For this review, take the finished solid that the model builds, in its own axes (mm). Face numbers are marked on the shaded views. A direction names the side the tool comes from. Round coordinates to 2 decimals unless told otherwise and drop trailing zeros. Write each loop counter-clockwise with the first axis right and the second up, starting at its lowest first coordinate (ties: lowest second). Pieces come first, ordered by that corner, then holes. Notation, with made-up numbers: (41.25, -30) -> (86.25, -30) arc R30 ccw to (86.25, 5) -> close; hole circle Ø5 at (45, -6). An arc over 180 degrees is marked (long way). Answer as CSV lines item,"result". Start each with the question number.
Item 1: Wall thickness on probe 1 along Y at (x, z) = (101.5, 18); probe 2 along Z at (x, y) = (75, -100); probe 3 along Y at (x, z) = (37, -8): over which ranges is each line inside the solid? List them lowest first. Write a range as from..to.
Item 2: For pin 1 Ø4 at (y, z) = (-101, -11.5) entering from -X; pin 2 Ø12 at (y, z) = (-50.5, -2) entering from -X; pin 3 Ø15 at (y, z) = (-28, 5.5) entering from +X; pin 4 Ø15 at (y, z) = (0, 0) entering from +X, all flat-tipped, find the tip position at first contact; note any pin that passes through.
Item 3: Take a section at B-B on x = 15. Give the boundary of the cut face in (y, z), then the cut area to 3 significant figures.
Item 4: Take a section at D-D on x = 79.5. Give the boundary of the cut face in (y, z), then the cut area to 3 significant figures.
Item 5: Machinability: for the marked faces 5, 6 and 7, which of the approach directions +Z, -Z, +X, -X, +Y, -Y give a long, thin tool a straight path to every point of the face, cutting with its end or side? Answer none if there is none.
Item 6: Take a section at C-C on y = -49. Give the boundary of the cut face in (x, z), then the cut area to 3 significant figures.
Item 7: Take a section at A-A on z = 0. Give the boundary of the cut face in (x, y), then the cut area to 3 significant figures.
Item 8: Mouldability with a two-part tool opening along Y and no side actions: class the marked faces 1, 2, 3 and 4 as +Y half, -Y half, draft (parallel to the pull), parting line (faces both ways), or undercut.
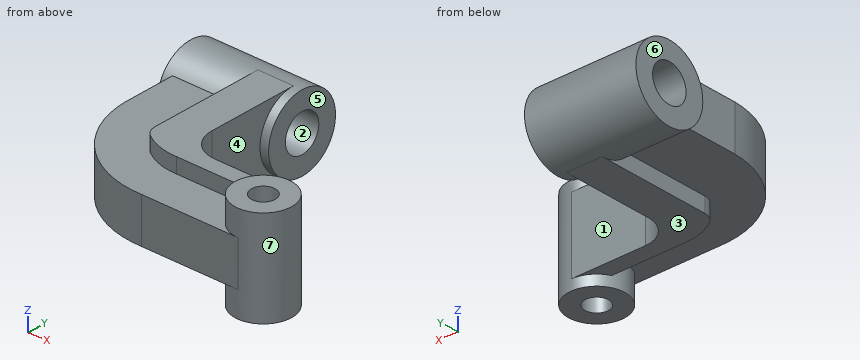
```python
from build123d import *

# Parameters (mm, degrees)
HUB_1_PROFILE_R       = 25
HUB_1_BOSS_75MM_DEPTH = 37.5
HUB_2_PROFILE_R       = 19
HUB_2_BOSS_64MM_DEPTH = 32
CURVED_ARM_WEB_DEPTH  = 15
ARM_FLANGE_DEPTH      = 25
HUB_1_BORE_PROFILE_R  = 12.5
HUB_1_BORE_DEPTH      = 88
HUB_2_BORE_PROFILE_R  = 8
HUB_2_BORE_DEPTH      = 88


with BuildPart() as part:
    # Hub 1 Profile → Hub 1 Boss 75mm (new, symmetric)
    with BuildSketch(Plane(origin=(0, 0, 0), x_dir=(0, 0, -1), z_dir=(1, 0, 0))):
        Circle(HUB_1_PROFILE_R)
    extrude(amount=HUB_1_BOSS_75MM_DEPTH, both=True)



with BuildPart() as body_2:
    # Hub 2 Profile → Hub 2 Boss 64mm (new, symmetric)
    with BuildSketch(Plane.XY):
        with Locations((101.5, -100)):
            Circle(HUB_2_PROFILE_R)
    extrude(amount=HUB_2_BOSS_64MM_DEPTH, both=True)


with BuildPart() as part_1:
    add(part.part)

    add(body_2.part)  # Curved Arm Web merges body 2
    # Curved Arm Profile → Curved Arm Web (add, symmetric)
    with BuildSketch(Plane.XY):
        with BuildLine():
            Line((36.70784585, -119), (101.5, -119))
            ThreePointArc((101.5, -119), (85.489542295, -110.23060331), (84.258248254, -92.017394113))
            Line((84.258248254, -92.017394113), (35.73883627, -92.017394113))
            ThreePointArc((35.73883627, -92.017394113), (23.331450339, -90.456826651), (12.055799796, -85.049581394))
            ThreePointArc((12.055799796, -85.049581394), (8.905598759, -81.472069365), (7.769480814, -76.842642304))
            Line((7.769480814, -76.842642304), (7.769480814, -18.704046106))
            Line((7.769480814, -18.704046106), (-31.61832529, -18.704046106))
            Line((-31.61832529, -18.704046106), (-31.61832529, -25))
            Line((-31.61832529, -25), (-31.61832529, -55.411209028))
            ThreePointArc((-31.61832529, -55.411209028), (-10.624909538, -101.356417889), (36.70784585, -119))
        make_face()
    extrude(amount=CURVED_ARM_WEB_DEPTH, both=True)

    # Arm Flange Profile → Arm Flange (add, symmetric)
    with BuildSketch(Plane.XY):
        with BuildLine():
            Line((31.704445688, -20), (31.704445688, -61))
            ThreePointArc((31.704445688, -61), (37.562310065, -75.142135624), (51.704445688, -81))
            Line((51.704445688, -81), (101.5, -81))
            ThreePointArc((101.5, -81), (91.26939669, -83.989542295), (84.258248254, -92.017394113))
            Line((84.258248254, -92.017394113), (35.73883627, -92.017394113))
            ThreePointArc((35.73883627, -92.017394113), (23.331450339, -90.456826651), (12.055799796, -85.049581394))
            ThreePointArc((12.055799796, -85.049581394), (8.905598759, -81.472069365), (7.769480814, -76.842642304))
            Line((7.769480814, -76.842642304), (7.769480814, -20))
            Line((7.769480814, -20), (7.769480814, 0))
            Line((7.769480814, 0), (31.704445688, 0))
            Line((31.704445688, 0), (31.704445688, -20))
        make_face()
    extrude(amount=ARM_FLANGE_DEPTH, both=True)

    # Hub 1 Bore Profile → Hub 1 Bore (cut)
    with BuildSketch(Plane(origin=(37.5, 0, 0), x_dir=(0, 0, -1), z_dir=(1, 0, 0))):
        Circle(HUB_1_BORE_PROFILE_R)
    extrude(amount=-HUB_1_BORE_DEPTH, mode=Mode.SUBTRACT)

    # Hub 2 Bore Profile → Hub 2 Bore (cut)
    with BuildSketch(Plane(origin=(0, 0, -32), x_dir=(-1, 0, 0), z_dir=(0, 0, -1))):
        with Locations((-101.5, -100)):
            Circle(HUB_2_BORE_PROFILE_R)
    extrude(amount=-HUB_2_BORE_DEPTH, mode=Mode.SUBTRACT)


solid = part_1.part
```
Output values:
1,probe 1,"y = -119..-108, -92..-81"
1,probe 2,"z = -15..15"
1,probe 3,"y = -119..-74.56, -23.69..-9.6, 9.6..23.69"
2,pin 1,"stops at x = -13.03"
2,pin 2,"stops at x = -31.62"
2,pin 3,"stops at x = 37.5"
2,pin 4,"passes through"
3,outline,"(-116.15, -15) -> (-86.91, -15) -> (-86.91, -25) -> (0, -25) arc R25 ccw to (0, 25) -> (-86.91, 25) -> (-86.91, 15) -> (-116.15, 15) -> close; hole circle Ø25 at (0, 0)"
3,area,"5,710 mm^2"
4,outline,"(-119, -15) -> (-92.02, -15) -> (-92.02, -25) -> (-81, -25) -> (-81, 25) -> (-92.02, 25) -> (-92.02, 15) -> (-119, 15) -> close"
4,area,"1,360 mm^2"
5,face 5,"+Z, -Z, +X, +Y"
5,face 6,"+Z, -Z, -X, +Y, -Y"
5,face 7,"none"
6,outline,"(-31.62, -15) -> (7.77, -15) -> (7.77, -25) -> (31.7, -25) -> (31.7, 25) -> (7.77, 25) -> (7.77, 15) -> (-31.62, 15) -> close"
6,area,"2,380 mm^2"
7,outline,"(-37.5, -25) -> (-31.62, -25) -> (-31.62, -55.41) arc R66 ccw to (36.71, -119) -> (101.5, -119) arc R19 ccw to (101.5, -81) -> (51.7, -81) arc R20 cw to (31.7, -61) -> (31.7, -25) -> (37.5, -25) -> (37.5, -12.5) -> (-37.5, -12.5) -> close; (-37.5, 12.5) -> (37.5, 12.5) -> (37.5, 25) -> (-37.5, 25) -> close; hole circle Ø16 at (101.5, -100)"
7,area,"10,000 mm^2"
8,face 1,"+Y half"
8,face 2,"undercut"
8,face 3,"draft"
8,face 4,"undercut"
